```python
from build123d import *

# Parameters (mm, degrees)
SKETCH1_W           = 232.3
SKETCH1_H           = 194
BOSS_EXTRUDE1_DEPTH = 3
SKETCH2_R           = 19
CUT_EXTRUDE1_DEPTH  = 3
SKETCH3_R           = 2
CUT_EXTRUDE2_DEPTH  = 4
SKETCH4_R           = 2
CUT_EXTRUDE3_DEPTH  = 152.356607058


with BuildPart() as part:
    # Sketch1 → Boss-Extrude1 (new body)
    with BuildSketch(Plane.XY):
        Rectangle(SKETCH1_W, SKETCH1_H)
    extrude(amount=BOSS_EXTRUDE1_DEPTH)

    # Sketch2 → Cut-Extrude1 (cut)
    with BuildSketch(Plane.XY.offset(3)):
        with Locations((0, -52)):
            Circle(SKETCH2_R)
    extrude(amount=-CUT_EXTRUDE1_DEPTH, mode=Mode.SUBTRACT)

    # Sketch3 → Cut-Extrude2 (cut)
    with BuildSketch(Plane.XY.offset(3)):
        with Locations((0, 92)):
            Circle(SKETCH3_R)
        with Locations((0, -92)):
            Circle(SKETCH3_R)
    extrude(amount=-CUT_EXTRUDE2_DEPTH, mode=Mode.SUBTRACT)

    # Sketch4 → Cut-Extrude3 (cut, through all)
    with BuildSketch(Plane.XY.offset(3)):
        with Locations((-113.15, 78)):
            Circle(SKETCH4_R)
        with Locations((-113.15, 28)):
            Circle(SKETCH4_R)
        with Locations((-113.15, -22)):
            Circle(SKETCH4_R)
        with Locations((-113.15, -42)):
            Circle(SKETCH4_R)
        with Locations((-113.15, -62)):
            Circle(SKETCH4_R)
    cut_extrude3 = extrude(amount=-CUT_EXTRUDE3_DEPTH, mode=Mode.SUBTRACT)

    # Mirror1: Cut-Extrude3 across plane
    add(cut_extrude3.mirror(Plane(origin=(0, 0, 0), x_dir=(0, 0, 1), z_dir=(1, 0, 0))), mode=Mode.SUBTRACT)


solid = part.part
```
Geometry: final body of the model. Coordinates: model frame, mm. Coordinates: 2 decimals unless noted, no trailing zeros. Order: outer loops, then holes, each group sorted by start corner. A loop starts at its lowest first (then second) coordinate and runs counter-clockwise, first axis right, second up. Notation, with made-up numbers: (31, 27) -> (55, 27) arc R20 cw to (55, 46) -> close; hole circle Ø2 at (-38.75, 8). An arc over 180 degrees is marked (long way). Use CSV: the item, a comma, the result in double quotes.
1) Section B-B on z = 1.15. State how many separate pieces and enclosed holes the cut face has, then the cut area to 3 significant figures.
Findings:
separate pieces,"1"
enclosed holes,"13"
area,"43,800 mm^2"
2) Line query: line 1 (Y direction, x = 113.15, z = 1.4); line 2 (X direction, y = -53.5, z = 0.2); line 3 (X direction, y = 79.5, z = 2.55). Output: solid intervals per line, ascending.
Findings:
line 1,"y = -97 to -64, -60 to -44, -40 to -24, -20 to 26, 30 to 76, 80 to 97"
line 2,"x = -116.15 to -18.94, 18.94 to 116.15"
line 3,"x = -116.15 to -114.47, -111.83 to 111.83, 114.47 to 116.15"
3) Section A-A on y = -52. Output: boundary loops of the cut face in (x, z).
Findings:
outline,"(-116.15, 0) -> (-19, 0) -> (-19, 3) -> (-116.15, 3) -> close; (19, 0) -> (116.15, 0) -> (116.15, 3) -> (19, 3) -> close"
4) Pin query (flat end, axial travel): pin 1 Ø3.5 at (x, y) = (-113.15, -42) entering from -Z. Return the tip coordinate at first contact, or that it passes through.
Findings:
pin 1,"passes through"
5) Section C-C on x = 5. Output: boundary loops of the cut face in (y, z).
Findings:
outline,"(-97, 0) -> (-70.33, 0) -> (-70.33, 3) -> (-97, 3) -> close; (-33.67, 0) -> (97, 0) -> (97, 3) -> (-33.67, 3) -> close"
6) Mould query, pull axis X, two halves, no side actions, for faces 1 (the flat face through (-2, 1, 3)), 2 (the cylindrical face through (18.12, -46.29, 1.52)). Classes: +X half, -X half, draft (parallel to the pull), parting line (faces both ways), or undercut.
Findings:
face 1,"draft"
face 2,"undercut"
